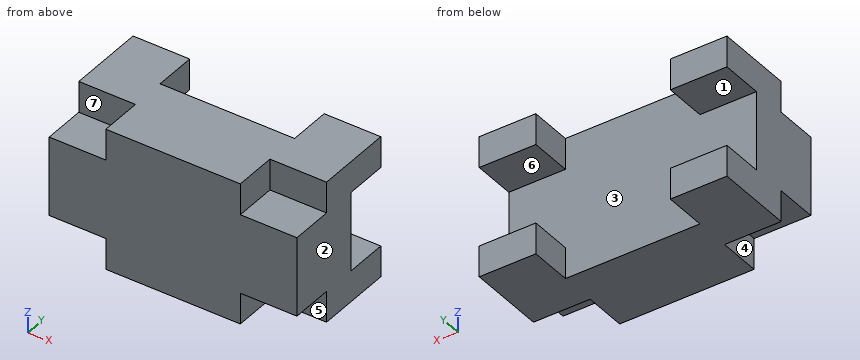
from build123d import *

# Parameters (mm, degrees)
BASE_PLATE_SKETCH_W         = 175
BASE_PLATE_SKETCH_H         = 100
BASE_PLATE_175X100X25_DEPTH = 25
TOP_BLOCKS_SKETCH_W         = 40
TOP_BLOCKS_SKETCH_H         = 22
TOP_BLOCKS_4X40X22_DEPTH    = 30
BOTTOM_PADS_DEPTH           = 30


with BuildPart() as part:
    # Base Plate Sketch → Base Plate 175x100x25 (new body)
    with BuildSketch(Plane(origin=(0, 0, 0), x_dir=(1, 0, 0), z_dir=(0, 1, 0))):
        Rectangle(BASE_PLATE_SKETCH_W, BASE_PLATE_SKETCH_H)
    extrude(amount=BASE_PLATE_175X100X25_DEPTH)

    # Top Blocks Sketch → Top Blocks 4x40x22 (add)
    with BuildSketch(Plane(origin=(0, 25, 0), x_dir=(1, 0, 0), z_dir=(0, 1, 0))):
        with Locations((-67.5, -39)):
            Rectangle(TOP_BLOCKS_SKETCH_W, TOP_BLOCKS_SKETCH_H)
        with Locations((-67.5, 39)):
            Rectangle(TOP_BLOCKS_SKETCH_W, TOP_BLOCKS_SKETCH_H)
        with Locations((67.5, 39)):
            Rectangle(TOP_BLOCKS_SKETCH_W, TOP_BLOCKS_SKETCH_H)
        with Locations((67.5, -39)):
            Rectangle(TOP_BLOCKS_SKETCH_W, TOP_BLOCKS_SKETCH_H)
    extrude(amount=TOP_BLOCKS_4X40X22_DEPTH)

    # Bottom Pads Sketch → Bottom Pads (add)
    with BuildSketch(Plane.XZ):
        Polygon((-47.5, 50), (47.5, 50), (47.5, 28), (87.5, 28), (87.5, -28), (47.5, -28), (47.5, -50), (-47.5, -50), (-47.5, -28), (-87.5, -28), (-87.5, 28), (-47.5, 28), align=None)
    extrude(amount=BOTTOM_PADS_DEPTH)


solid = part.part
Build history of the part. All positions in model axes, mm. Face numbers are marked on the shaded views. A direction names the side the tool comes from. Coordinates: 2 decimals unless noted, no trailing zeros. Order: outer loops, then holes, each group sorted by start corner. A loop starts at its lowest first (then second) coordinate and runs counter-clockwise, first axis right, second up. Notation, with made-up numbers: (68, 86) - (91, 86) arc R24 ccw to (91, 109) - close; hole circle Ø5 at (62.25, 32.25). An arc over 180 degrees is marked (long way). Write item = value, one per line. Start each with the question number.
1) Two-plate mould, pull along X, no slides. Class the marked faces 1, 2, 3 and 4: pulls with the +X half, pulls with the -X half, needs draft (parallel to the pull), parting line crosses it, or undercut.
2) Flat gauge pins, fed straight in: pin 1 Ø6.5 at (x, z) = (-64, -44.5) entering from -Y; pin 2 Ø11 at (y, z) = (-15, 41) entering from +X; pin 3 Ø24 at (x, y) = (69.5, -18.5) entering from +Z. Where does each tip first touch, or does it go through?
3) Wall check: line 1 along X through (y, z) = (37, 38); line 2 along Z through (x, y) = (78, 51); line 3 along Y through (x, z) = (-28, 32.5). Give the ranges that are in metal, low to high. Write a range as from..to.
4) Saw through at D-D on z = -4. Write the cut outline in (x, y), then the cut area to 4 significant figures.
5) Saw through at A-A on y = 45. Write the cut outline in (x, z), then the cut area to 3 significant figures.
6) 3-axis set-ups, long thin cutter, end or side, ignore diameter. For the marked faces 5, 6 and 7: which of +Z, -Z, +X, -X, +Y, -Y reach the whole face in a straight line?
7) Saw through at C-C on x = 31.5. Write the cut outline in (y, z).
8) Saw through at B-B on y = -2. Write the cut outline in (x, z).
From the geometry:
q1.face_1 = needs draft
q1.face_2 = pulls with the +X half
q1.face_3 = undercut
q1.face_4 = pulls with the -X half
q2.pin_1 = 0
q2.pin_2 = 47.5
q2.pin_3 = 28
q3.line_1 = -87.5..-47.5, 47.5..87.5
q3.line_2 = -50..-28, 28..50
q3.line_3 = -30..25
q4.outline = (-87.5, -30) - (87.5, -30) - (87.5, 25) - (-87.5, 25) - close
q4.area = 9,625 mm^2
q5.outline = (-87.5, -50) - (-47.5, -50) - (-47.5, -28) - (-87.5, -28) - close; (-87.5, 28) - (-47.5, 28) - (-47.5, 50) - (-87.5, 50) - close; (47.5, -50) - (87.5, -50) - (87.5, -28) - (47.5, -28) - close; (47.5, 28) - (87.5, 28) - (87.5, 50) - (47.5, 50) - close
q5.area = 3,520 mm^2
q6.face_5 = -Z, +X, -Y
q6.face_6 = +X, -X, +Y
q6.face_7 = +Z, -X, -Y
q7.outline = (-30, -50) - (25, -50) - (25, 50) - (-30, 50) - close
q8.outline = (-87.5, -28) - (-47.5, -28) - (-47.5, -50) - (47.5, -50) - (47.5, -28) - (87.5, -28) - (87.5, 28) - (47.5, 28) - (47.5, 50) - (-47.5, 50) - (-47.5, 28) - (-87.5, 28) - close
